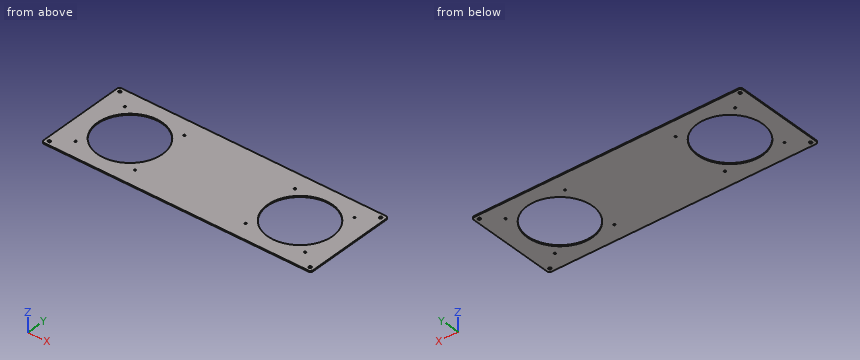
```python
from build123d import *

# Parameters (mm, degrees)
SKETCH_1_W             = 475
SKETCH_1_H             = 165
EXTRUDE_1_DEPTH        = 2
HOLE_WIZARD_5_0_5_1_D  = 5
CHAMFER_1_SIZE         = 3
SKETCH_4_R             = 57.5
CUT_EXTRUDE_1_DEPTH    = 2
HOLE_WIZARD_M4_1_D     = 3.3
HOLE_WIZARD_M4_1_DEPTH = 10.1
HOLE_WIZARD_M4_1_TIP   = 0.991420021


with BuildPart() as part:
    # 草图1 → 凸台-拉伸1 (new body)
    with BuildSketch(Plane.XY):
        Rectangle(SKETCH_1_W, SKETCH_1_H)
    extrude(amount=EXTRUDE_1_DEPTH)

    # Ø5.0 (5) 直径孔1 (through all)
    with Locations(Plane.XY.offset(2)):
        with Locations((-230, 75), (-230, -75), (230, 75), (230, -75)):
            Hole(HOLE_WIZARD_5_0_5_1_D / 2)

    # 倒角1
    chamfer_1_edges = [part.edges().sort_by_distance(p)[0] for p in [
        (237.5, -82.5, 1),
        (-237.5, -82.5, 1),
        (-237.5, 82.5, 1),
        (237.5, 82.5, 1),
    ]]
    chamfer(chamfer_1_edges, length=CHAMFER_1_SIZE)

    # 草图4 → 切除-拉伸1 (cut)
    with BuildSketch(Plane.XY.offset(2)):
        with Locations((-150, 0)):
            Circle(SKETCH_4_R)
        with Locations((150, 0)):
            Circle(SKETCH_4_R)
    extrude(amount=-CUT_EXTRUDE_1_DEPTH, mode=Mode.SUBTRACT)

    # M4 螺纹孔1
    with Locations(Plane.XY.offset(2)):
        with Locations((-202.5, 52.5), (-97.5, 52.5), (-97.5, -52.5), (-202.5, -52.5), (97.5, -52.5), (202.5, -52.5), (202.5, 52.5), (97.5, 52.5)):
            Hole(HOLE_WIZARD_M4_1_D / 2, depth=HOLE_WIZARD_M4_1_DEPTH)
            with Locations((0, 0, -(HOLE_WIZARD_M4_1_DEPTH + HOLE_WIZARD_M4_1_TIP / 2))):  # 118° drill point
                Cone(0, HOLE_WIZARD_M4_1_D / 2, HOLE_WIZARD_M4_1_TIP, mode=Mode.SUBTRACT)


solid = part.part
```
Work out the finished part from the listing and answer in its coordinate system (mm). Coordinates: 2 decimals unless noted, no trailing zeros. Loops run counter-clockwise (first coordinate to the right, second up) from the corner with the lowest first, then second, coordinate; pieces in that order, holes last. Notation, with made-up numbers: M 62,30 L 106,30 A20 cw 106,41 Z; hole C -3,61 d3. An arc over 180 degrees is marked long. Use CSV: the item, a comma, the result in double quotes. Start each with the question number.
(1) Find section B-B, the plane z = 1.3. State how many separate pieces and enclosed holes the cut face has, then the cut area to 3 significant figures.
(2) Find section D-D, the plane y = 40.5. Give the vertices of the cut face in (x, z).
(3) Find section C-C, the plane x = 162.5. Give the vertices of the cut face in (y, z), then the cut area to 3 significant figures.
(4) Consider line 1 (X direction, y = -2, z = 1); line 2 (Y direction, x = 230, z = 0.5); line 3 (X direction, y = -32, z = 1.6). Determine where each line is inside the solid, lowest interval first.
(5) Find section A-A, the plane y = 0. Give the vertices of the cut face in (x, z).
Recorded:
1,separate pieces,"1"
1,enclosed holes,"14"
1,area,"57,400 mm^2"
2,outline,"M -237.5,0 L -190.82,0 L -190.82,2 L -237.5,2 Z; M -109.18,0 L 109.18,0 L 109.18,2 L -109.18,2 Z; M 190.82,0 L 237.5,0 L 237.5,2 L 190.82,2 Z"
3,outline,"M -82.5,0 L -56.12,0 L -56.12,2 L -82.5,2 Z; M 56.12,0 L 82.5,0 L 82.5,2 L 56.12,2 Z"
3,area,"106 mm^2"
4,line 1,"x = -237.5 to -207.47, -92.53 to 92.53, 207.47 to 237.5"
4,line 2,"y = -82.5 to -77.5, -72.5 to 72.5, 77.5 to 82.5"
4,line 3,"x = -237.5 to -197.77, -102.23 to 102.23, 197.77 to 237.5"
5,outline,"M -237.5,0 L -207.5,0 L -207.5,2 L -237.5,2 Z; M -92.5,0 L 92.5,0 L 92.5,2 L -92.5,2 Z; M 207.5,0 L 237.5,0 L 237.5,2 L 207.5,2 Z"
